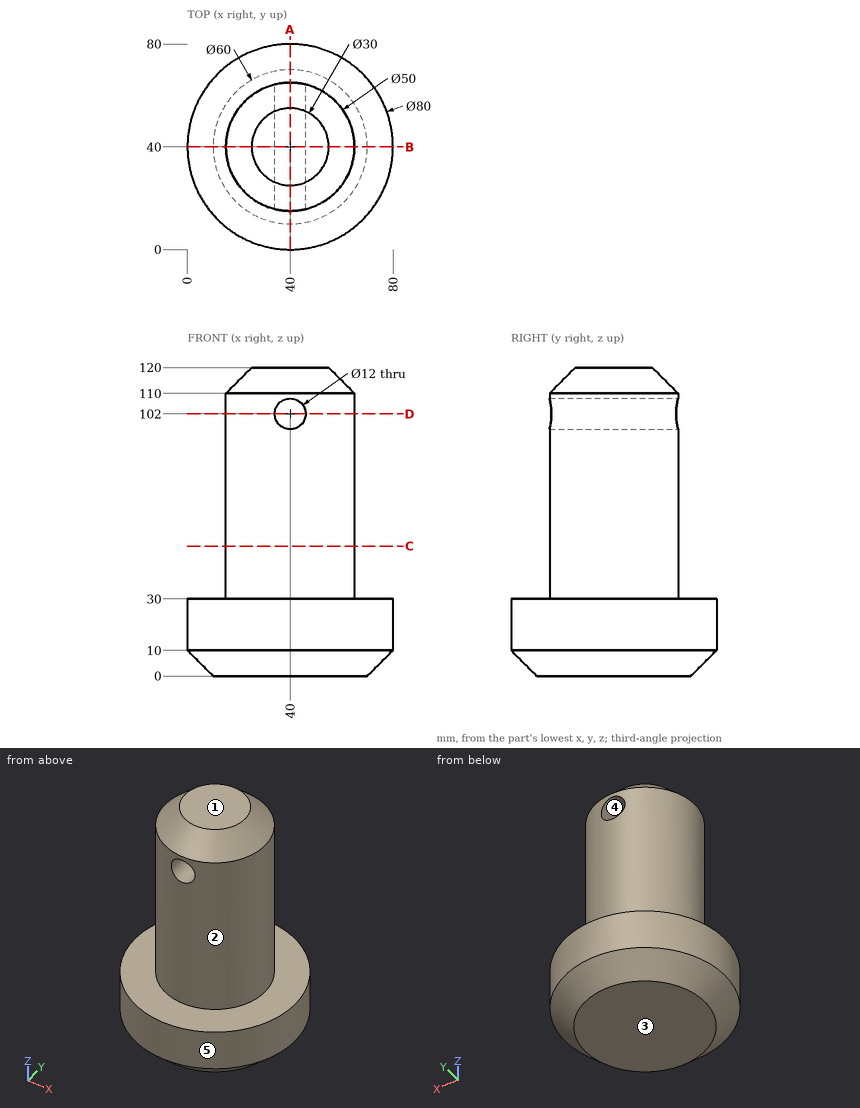
Input: dimensioned drawing with shaded views. Units: mm. Origin: part minimum x, y, z. A direction names the side the tool comes from. Coordinates: 2 decimals unless noted, no trailing zeros. Write each loop counter-clockwise with the first axis right and the second up, starting at its lowest first coordinate (ties: lowest second). Pieces come first, ordered by that corner, then holes. Notation, with made-up numbers: M -19.75,-36.5 L 20.25,-36.5 A26 ccw 20.25,-12.5 Z; hole C -15,33 d6. An arc over 180 degrees is marked long. Answer as CSV lines item,"result". Start each with the question number.
Q1. Cut plane D-D on z = 102. Return the cut outline in (x, y), then the cut area to 3 significant figures.
Q2. Mould query, pull axis Z, two halves, no side actions, for the marked faces 3, 4 and 5. Classes: released by +Z, released by -Z, zero draft, split by the parting line, or undercut.
Q3. Cut plane A-A on x = 40. Return the cut outline in (y, z), then the cut area to 3 significant figures.
Q4. Line query: line 1 (Z direction, x = 40, y = 32); line 2 (X direction, y = 36.5, z = 102); line 3 (X direction, y = 44.5, z = 102). Output: solid intervals per line, ascending. Write a range as from..to.
Q5. Cut plane B-B on y = 40. Return the cut outline in (x, z), then the cut area to 3 significant figures.
Q6. Pin query (flat end, axial travel): P1, Ø24, axis at x = 43, y = 23.5, coming from the +Z side; P2, Ø2, axis at y = 43, z = 27, coming from the -X side; P3, Ø19, axis at x = 40, z = 102, coming from the +Y side; P4, Ø8, axis at x = 15.5, y = 49, coming from the +Z side. Return the tip coordinate at first contact, or that it passes through.
Q7. Reachability of the marked faces 1 and 2 from +Z, -Z, +X, -X, +Y, -Y: full face, straight path, thin tool, end or side. Return the list, or none.
Q8. Cut plane C-C on z = 50.5. Return the cut outline in (x, y), then the cut area to 3 significant figures.
Findings below:
1,outline,"M 34,15.73 L 34,64.27 A25 ccw Z; M 46,15.73 A25 ccw 46,64.27 Z"
1,area,"1,370 mm2"
2,face 3,"released by -Z"
2,face 4,"undercut"
2,face 5,"zero draft"
3,outline,"M 0,10 L 10,0 L 70,0 L 80,10 L 80,30 L 65,30 L 65,96 L 15,96 L 15,30 L 0,30 Z; M 15,108 L 65,108 L 65,110 L 55,120 L 25,120 L 15,110 Z"
3,area,"6,100 mm2"
4,line 1,"z = 0..96, 108..120"
4,line 2,"x = 15.25..34, 46..64.75"
4,line 3,"x = 15.41..34, 46..64.59"
5,outline,"M 0,10 L 10,0 L 70,0 L 80,10 L 80,30 L 65,30 L 65,110 L 55,120 L 25,120 L 15,110 L 15,30 L 0,30 Z; hole C 40,102 d12"
5,area,"6,590 mm2"
6,P1,"stops at z = 120"
6,P2,"stops at x = 0.05"
6,P3,"stops at y = 65"
6,P4,"stops at z = 112.9"
7,face 1,"+Z, +X, -X, +Y, -Y"
7,face 2,"+Z"
8,outline,"C 40,40 d50"
8,area,"1,960 mm2"
